CAD build for the part. Positions are in the model's coordinates, mm. A direction names the side the tool comes from. Coordinates: 2 decimals unless noted, no trailing zeros. Order: outer loops, then holes, each group sorted by start corner. A loop starts at its lowest first (then second) coordinate and runs counter-clockwise, first axis right, second up.
from build123d import *

# Parameters (mm, degrees)
SKETCH_1_W                = 130
SKETCH_1_H                = 50
EXTRUDE_1_DEPTH           = 15.35
CHAMFER_1_SIZE            = 2
HOLE_WIZARD_M12_1_D       = 10.2
HOLE_WIZARD_1_D           = 6.6
HOLE_WIZARD_1_CBORE_D     = 11
HOLE_WIZARD_1_CBORE_DEPTH = 6.8


with BuildPart() as part:
    # 草图1 → 凸台-拉伸1 (new, symmetric)
    with BuildSketch(Plane(origin=(0, 0, 0), x_dir=(1, 0, 0), z_dir=(0, 1, 0))):
        Rectangle(SKETCH_1_W, SKETCH_1_H)
    extrude(amount=EXTRUDE_1_DEPTH, both=True)

    # 倒角1
    chamfer_1_edges = [part.edges().sort_by_distance(p)[0] for p in [
        (65, 0, 25),
        (-65, 0, 25),
        (-65, 0, -25),
        (65, 0, -25),
    ]]
    chamfer(chamfer_1_edges, length=CHAMFER_1_SIZE)

    # M12 螺纹孔1 (through all)
    with Locations(Plane(origin=(0, 15.35, 0), x_dir=(1, 0, 0), z_dir=(0, 1, 0))):
        with Locations((-47.5, 0), (47.5, 0)):
            Hole(HOLE_WIZARD_M12_1_D / 2)

    # 打孔尺寸(%根据)内六角圆柱头螺钉的类型1 (through all)
    with Locations(Plane(origin=(0, 15.35, 0), x_dir=(1, 0, 0), z_dir=(0, 1, 0))):
        with Locations((-5, -15), (-5, 15)):
            CounterBoreHole(HOLE_WIZARD_1_D / 2, HOLE_WIZARD_1_CBORE_D / 2, HOLE_WIZARD_1_CBORE_DEPTH)


solid = part.part
1) Drill centre lines: probe 1 along Z at (x, y) = (-5, 12); probe 2 along Z at (x, y) = (-5, -7.5); probe 3 along X at (y, z) = (-10, -15). Where is each one in solid material? Low to high.
2) Slice it at C-C (x = -5). List the corners of the cut face in (y, z), plus the area to 3 significant figures.
3) Two-plate mould, pull along X, no slides. Class faces 1 (the flat face through (65, 0, 0)), 2 (the flat face through (-65, 0, 0)), 3 (the cylindrical face through (-42.405, -0.215, -0.224)): released by +X, released by -X, zero draft, split by the parting line, or undercut.
4) Slice it at A-A (z = -15). List the corners of the cut face in (x, y).
5) Slice it at B-B (y = -5). List the corners of the cut face in (x, z).
6) Slice it at D-D (z = 0). List the corners of the cut face in (x, y).
7) Which spindle directions (+Z, -Z, +X, -X, +Y, -Y) get a long thin tool onto all of the face, cutting with end or side? Do faces 4 (the cylindrical face through (52.595, -0.215, -0.224)), 5 (the cylindrical face through (-6.19, 12, 20.37)). Say none if no direction does.
Worked out:
1. probe 1: z = -25 to -20.5, -9.5 to 9.5, 20.5 to 25
1. probe 2: z = -25 to -18.3, -11.7 to 11.7, 18.3 to 25
1. probe 3: x = -65 to -8.3, -1.7 to 65
2. outline: (-15.35, -25) - (15.35, -25) - (15.35, -20.5) - (8.55, -20.5) - (8.55, -18.3) - (-15.35, -18.3) - close; (-15.35, -11.7) - (8.55, -11.7) - (8.55, -9.5) - (15.35, -9.5) - (15.35, 9.5) - (8.55, 9.5) - (8.55, 11.7) - (-15.35, 11.7) - close; (-15.35, 18.3) - (8.55, 18.3) - (8.55, 20.5) - (15.35, 20.5) - (15.35, 25) - (-15.35, 25) - close
2. area: 1,070 mm2
3. face 1: released by +X
3. face 2: released by -X
3. face 3: undercut
4. outline: (-65, -15.35) - (-8.3, -15.35) - (-8.3, 8.55) - (-10.5, 8.55) - (-10.5, 15.35) - (-65, 15.35) - close; (-1.7, -15.35) - (65, -15.35) - (65, 15.35) - (0.5, 15.35) - (0.5, 8.55) - (-1.7, 8.55) - close
5. outline: (-65, -23) - (-63, -25) - (63, -25) - (65, -23) - (65, 23) - (63, 25) - (-63, 25) - (-65, 23) - close; hole circle Ø10.2 at (-47.5, 0); hole circle Ø6.6 at (-5, -15); hole circle Ø6.6 at (-5, 15); hole circle Ø10.2 at (47.5, 0)
6. outline: (-65, -15.35) - (-52.6, -15.35) - (-52.6, 15.35) - (-65, 15.35) - close; (-42.4, -15.35) - (42.4, -15.35) - (42.4, 15.35) - (-42.4, 15.35) - close; (52.6, -15.35) - (65, -15.35) - (65, 15.35) - (52.6, 15.35) - close
7. face 4: +Y, -Y
7. face 5: +Y
